The model under review builds one solid part; all positions refer to its coordinate system, in mm. Face numbers are marked on the shaded views. A direction names the side the tool comes from. Coordinates: 2 decimals unless noted, no trailing zeros. Loops run counter-clockwise (first coordinate to the right, second up) from the corner with the lowest first, then second, coordinate; pieces in that order, holes last. Notation, with made-up numbers: (80.25, 56) - (132.25, 56) arc R25 cw to (132.25, 74) - close; hole circle Ø1 at (12, 4). An arc over 180 degrees is marked (long way). One line per item, written item: value. Start each with the question number.
1. We need section D-D, the plane x = 0. Give the boundary of the cut face in (y, z), then the cut area to 3 significant figures.
2. For the marked faces 1, 2 and 3, list the 3-axis set-ups (+Z, -Z, +X, -X, +Y, -Y) from which the entire face can be reached by the end or side of a thin tool; tool diameter is ignored.
3. We need section B-B, the plane z = -9. Give the boundary of the cut face in (x, y), then the cut area to 3 significant figures.
4. To check wall thickness, follow line 1 (X direction, y = 92, z = -17); line 2 (X direction, y = 75, z = -6); line 3 (Y direction, x = -18, z = -2.5). State the ranges of each line that lie inside material, in increasing order.
5. Insertion check: P1, Ø2, axis at y = 73, z = -8.5, coming from the +X side; P2, Ø4, axis at x = 18, z = -17.5, coming from the -Y side; P3, Ø11, axis at x = 25.5, z = -1, coming from the +Y side. Each pin has a flat end and moves straight along its axis. Give the tip position at first contact, or say it passes through.
6. We need section C-C, the plane y = 82. Give the boundary of the cut face in (x, z), then the cut area to 3 significant figures.
7. We need section A-A, the plane x = 22.5. Give the boundary of the cut face in (y, z), then the cut area to 3 significant figures.
8. Mouldability with a two-part tool opening along Y and no side actions: class the marked faces 4, 5 and 6 as +Y half, -Y half, draft (parallel to the pull), parting line (faces both ways), or undercut.
from build123d import *

# Parameters (mm, degrees)
SKETCH1_W           = 42
SKETCH1_H           = 42
BOSS_EXTRUDE1_DEPTH = 95
SKETCH2_W           = 8
SKETCH2_H           = 8
CUT_EXTRUDE1_DEPTH  = 90.2
SKETCH3_R           = 1.8
CUT_EXTRUDE2_DEPTH  = 4.8
FILLET1_R           = 4
SKETCH4_R           = 15
BOSS_EXTRUDE2_DEPTH = 1.5
SKETCH5_R           = 4
BOSS_EXTRUDE3_DEPTH = 21
FILLET2_R           = 3
SKETCH8_W           = 21
SKETCH8_H           = 18
BOSS_EXTRUDE5_DEPTH = 10
SKETCH9_W           = 13.716177762
SKETCH9_H           = 4.011335006
CUT_EXTRUDE3_DEPTH  = 15


with BuildPart() as part:
    # Sketch1 → Boss-Extrude1 (new body)
    with BuildSketch(Plane(origin=(0, 0, 0), x_dir=(1, 0, 0), z_dir=(0, 1, 0))):
        Rectangle(SKETCH1_W, SKETCH1_H)
    extrude(amount=BOSS_EXTRUDE1_DEPTH)

    # Sketch2 → Cut-Extrude1 (cut)
    with BuildSketch(Plane.XZ):
        with Locations((-17, 17)):
            Rectangle(SKETCH2_W, SKETCH2_H)
        with Locations((17, 17)):
            Rectangle(SKETCH2_W, SKETCH2_H)
        with Locations((-17, -17)):
            Rectangle(SKETCH2_W, SKETCH2_H)
        with Locations((17, -17)):
            Rectangle(SKETCH2_W, SKETCH2_H)
    extrude(amount=-CUT_EXTRUDE1_DEPTH, mode=Mode.SUBTRACT)

    # Sketch3 → Cut-Extrude2 (cut)
    with BuildSketch(Plane(origin=(0, 95, 0), x_dir=(1, 0, 0), z_dir=(0, 1, 0))):
        with Locations(Location((-17, 17, 0), (0, 0, 270))):
            Circle(SKETCH3_R)
        with Locations(Location((17, 17, 0), (0, 0, 270))):
            Circle(SKETCH3_R)
        with Locations(Location((-17, -17, 0), (0, 0, 270))):
            Circle(SKETCH3_R)
        with Locations(Location((17, -17, 0), (0, 0, 270))):
            Circle(SKETCH3_R)
    extrude(amount=-CUT_EXTRUDE2_DEPTH, mode=Mode.SUBTRACT)

    # Fillet1
    fillet1_edges = [part.edges().sort_by_distance(p)[0] for p in [
        (-13, 45.1, 13),
        (13, 45.1, 13),
        (-13, 45.1, -13),
        (13, 45.1, -13),
    ]]
    fillet(fillet1_edges, radius=FILLET1_R)

    # Sketch4 → Boss-Extrude2 (add)
    with BuildSketch(Plane(origin=(0, 95, 0), x_dir=(1, 0, 0), z_dir=(0, 1, 0))):
        with Locations(Location((0, 0, 0), (0, 0, 90))):
            Circle(SKETCH4_R)
    extrude(amount=BOSS_EXTRUDE2_DEPTH)

    # Sketch5 → Boss-Extrude3 (add)
    with BuildSketch(Plane(origin=(0, 95, 0), x_dir=(1, 0, 0), z_dir=(0, 1, 0))):
        with Locations(Location((0, 0, 0), (0, 0, 90))):
            Circle(SKETCH5_R)
    extrude(amount=BOSS_EXTRUDE3_DEPTH)

    # Fillet2
    fillet2_edges = [part.edges().sort_by_distance(p)[0] for p in [
        (21, 92.6, 21),
        (-21, 92.6, 21),
        (-21, 92.6, -21),
        (21, 92.6, -21),
    ]]
    fillet(fillet2_edges, radius=FILLET2_R)

    # Sketch8 → Boss-Extrude5 (add)
    with BuildSketch(Plane(origin=(21, 0, 0), x_dir=(0, 0, -1), z_dir=(1, 0, 0))):
        with Locations((0, 9)):
            Rectangle(SKETCH8_W, SKETCH8_H)
        with Locations((0, 36)):
            Rectangle(SKETCH8_W, SKETCH8_H)
    extrude(amount=BOSS_EXTRUDE5_DEPTH)

    # Sketch9 → Cut-Extrude3 (cut)
    with BuildSketch(Plane(origin=(0, 116, 0), x_dir=(1, 0, 0), z_dir=(0, 1, 0))):
        with Locations((-1.407114482, -5.505667503)):
            Rectangle(SKETCH9_W, SKETCH9_H)
    extrude(amount=-CUT_EXTRUDE3_DEPTH, mode=Mode.SUBTRACT)


solid = part.part
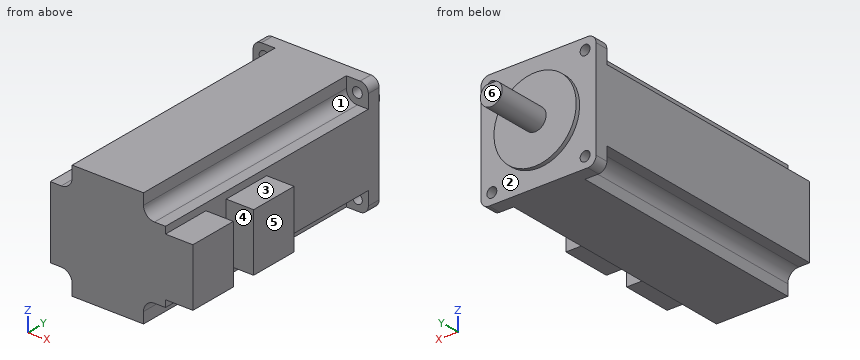
Findings below:
1. outline: (0, -21) - (95, -21) - (95, -15) - (96.5, -15) - (96.5, -4) - (116, -4) - (116, 3.5) - (101, 3.5) - (101, 4) - (96.5, 4) - (96.5, 15) - (95, 15) - (95, 21) - (0, 21) - close
1. area: 4,180 mm2
2. face 1: +Z, +X, -Y
2. face 2: +Y
2. face 3: +Z, +X, +Y, -Y
3. outline: (-21, 0) - (31, 0) - (31, 18) - (21, 18) - (21, 27) - (31, 27) - (31, 45) - (21, 45) - (21, 95) - (12, 95) - (12, 96.5) - (-12, 96.5) - (-12, 95) - (-21, 95) - close
3. area: 4,390 mm2
4. line 1: -21 to -18.8, -15.2 to 15.2, 18.8 to 21
4. line 2: -21 to 21
4. line 3: 0 to 95
5. P1: x = 21
5. P2: y = 90.2
5. P3: y = 95
6. outline: (-21, -13) - (-17, -13) arc R4 cw to (-13, -17) - (-13, -21) - (13, -21) - (13, -17) arc R4 cw to (17, -13) - (21, -13) - (21, 13) - (17, 13) arc R4 cw to (13, 17) - (13, 21) - (-13, 21) - (-13, 17) arc R4 cw to (-17, 13) - (-21, 13) - close
6. area: 1,520 mm2
7. outline: (0, -10.5) - (18, -10.5) - (18, 10.5) - (0, 10.5) - close; (27, -10.5) - (45, -10.5) - (45, 10.5) - (27, 10.5) - close
7. area: 756 mm2
8. face 4: undercut
8. face 5: draft
8. face 6: +Y half
